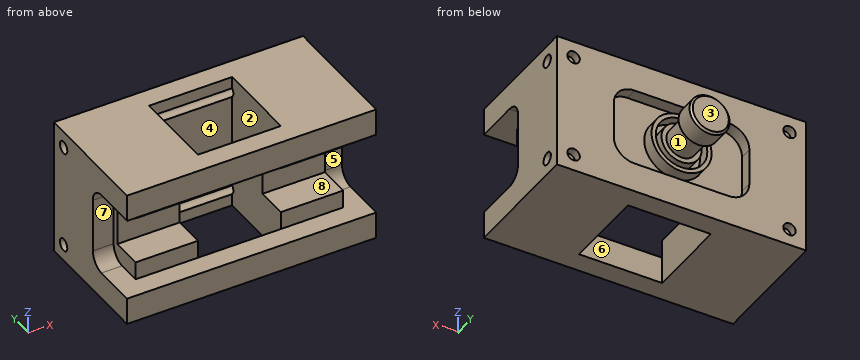
```python
from build123d import *

# Parameters (mm, degrees)
SKETCH1_W           = 120
SKETCH1_H           = 66
BOSS_EXTRUDE1_DEPTH = 60
SKETCH3_W           = 40
SKETCH3_H           = 20
CUT_EXTRUDE1_DEPTH  = 120
SKETCH4_W           = 40
SKETCH4_H           = 40
CUT_EXTRUDE2_DEPTH  = 120
SKETCH5_W           = 22.599154532
SKETCH5_H           = 30
CUT_EXTRUDE3_DEPTH  = 120
SKETCH6_R           = 3
CUT_EXTRUDE4_DEPTH  = 120
SKETCH7_W           = 40
SKETCH7_H           = 18
CUT_EXTRUDE5_DEPTH  = 10
SKETCH8_W           = 40
SKETCH8_H           = 18
CUT_EXTRUDE6_DEPTH  = 10
SKETCH9_W           = 65.307661508
SKETCH9_H           = 37.522692198
CUT_EXTRUDE7_DEPTH  = 6
FILLET1_R           = 10
SKETCH10_R          = 3
CUT_EXTRUDE8_DEPTH  = 4
FILLET2_R           = 7
SKETCH11_R          = 14.45708456
SKETCH11_R_2        = 12.407691548
BOSS_EXTRUDE2_DEPTH = 6
SKETCH12_R          = 9.667792976
BOSS_EXTRUDE3_DEPTH = 6
SKETCH13_R          = 7.310717913
BOSS_EXTRUDE4_DEPTH = 12
SKETCH14_R          = 9.667792976
BOSS_EXTRUDE5_DEPTH = 12
CHAMFER1_SIZE       = 2
CHAMFER2_SIZE       = 1


with BuildPart() as part:
    # Sketch1 → Boss-Extrude1 (new body)
    with BuildSketch(Plane(origin=(0, 0, 0), x_dir=(1, 0, 0), z_dir=(0, 1, 0))):
        Rectangle(SKETCH1_W, SKETCH1_H)
    extrude(amount=BOSS_EXTRUDE1_DEPTH)

    # Sketch3 → Cut-Extrude1 (cut)
    with BuildSketch(Plane(origin=(60, 0, 0), x_dir=(0, 0, -1), z_dir=(1, 0, 0))):
        Rectangle(SKETCH3_W, SKETCH3_H)
    extrude(amount=-CUT_EXTRUDE1_DEPTH, mode=Mode.SUBTRACT)

    # Sketch4 → Cut-Extrude2 (cut)
    with BuildSketch(Plane.XY.offset(33)):
        with Locations((0, 30)):
            Rectangle(SKETCH4_W, SKETCH4_H)
    extrude(amount=-CUT_EXTRUDE2_DEPTH, mode=Mode.SUBTRACT)

    # Sketch5 → Cut-Extrude3 (cut)
    with BuildSketch(Plane(origin=(60, 0, 0), x_dir=(0, 0, -1), z_dir=(1, 0, 0))):
        with Locations((0, 10)):
            Rectangle(SKETCH5_W, SKETCH5_H)
    extrude(amount=-CUT_EXTRUDE3_DEPTH, mode=Mode.SUBTRACT)

    # Sketch6 → Cut-Extrude4 (cut)
    with BuildSketch(Plane(origin=(60, 0, 0), x_dir=(0, 0, -1), z_dir=(1, 0, 0))):
        with Locations((-25, 52)):
            Circle(SKETCH6_R)
        with Locations((25, 52)):
            Circle(SKETCH6_R)
    extrude(amount=-CUT_EXTRUDE4_DEPTH, mode=Mode.SUBTRACT)

    # Sketch7 → Cut-Extrude5 (cut)
    with BuildSketch(Plane(origin=(60, 0, 0), x_dir=(0, 0, -1), z_dir=(1, 0, 0))):
        with Locations((0, 19)):
            Rectangle(SKETCH7_W, SKETCH7_H)
    extrude(amount=-CUT_EXTRUDE5_DEPTH, mode=Mode.SUBTRACT)

    # Sketch8 → Cut-Extrude6 (cut)
    with BuildSketch(Plane.ZY.offset(60)):
        with Locations((0, 19)):
            Rectangle(SKETCH8_W, SKETCH8_H)
    extrude(amount=-CUT_EXTRUDE6_DEPTH, mode=Mode.SUBTRACT)

    # Sketch9 → Cut-Extrude7 (cut)
    with BuildSketch(Plane(origin=(0, 60, 0), x_dir=(1, 0, 0), z_dir=(0, 1, 0))):
        Rectangle(SKETCH9_W, SKETCH9_H)
    extrude(amount=-CUT_EXTRUDE7_DEPTH, mode=Mode.SUBTRACT)

    # Fillet1
    fillet1_edges = [part.edges().sort_by_distance(p)[0] for p in [
        (32.653830754, 57, -18.761346099),
        (32.653830754, 57, 18.761346099),
        (-32.653830754, 57, 18.761346099),
        (-32.653830754, 57, -18.761346099),
    ]]
    fillet(fillet1_edges, radius=FILLET1_R)

    # Sketch10 → Cut-Extrude8 (cut)
    with BuildSketch(Plane(origin=(0, 60, 0), x_dir=(1, 0, 0), z_dir=(0, 1, 0))):
        with Locations(Location((-52, 25, 0), (0, 0, 270))):
            Circle(SKETCH10_R)
        with Locations(Location((52, 25, 0), (0, 0, 270))):
            Circle(SKETCH10_R)
        with Locations(Location((-52, -25, 0), (0, 0, 270))):
            Circle(SKETCH10_R)
        with Locations(Location((52, -25, 0), (0, 0, 270))):
            Circle(SKETCH10_R)
    extrude(amount=-CUT_EXTRUDE8_DEPTH, mode=Mode.SUBTRACT)

    # Fillet2
    fillet2_edges = [part.edges().sort_by_distance(p)[0] for p in [
        (55, 28, 20),
        (55, 28, -20),
        (-55, 28, -20),
        (-55, 28, 20),
    ]]
    fillet(fillet2_edges, radius=FILLET2_R)

    # Sketch11 → Boss-Extrude2 (add)
    with BuildSketch(Plane(origin=(0, 54, 0), x_dir=(1, 0, 0), z_dir=(0, 1, 0))):
        with Locations(Location((0, 0, 0), (0, 0, 270))):
            Circle(SKETCH11_R)
        with Locations(Location((0, 0, 0), (0, 0, 270))):
            Circle(SKETCH11_R_2, mode=Mode.SUBTRACT)
    extrude(amount=BOSS_EXTRUDE2_DEPTH)

    # Sketch12 → Boss-Extrude3 (add)
    with BuildSketch(Plane(origin=(0, 54, 0), x_dir=(1, 0, 0), z_dir=(0, 1, 0))):
        with Locations(Location((0, 0, 0), (0, 0, 270))):
            Circle(SKETCH12_R)
    extrude(amount=BOSS_EXTRUDE3_DEPTH)

    # Sketch13 → Boss-Extrude4 (add)
    with BuildSketch(Plane(origin=(0, 60, 0), x_dir=(1, 0, 0), z_dir=(0, 1, 0))):
        with Locations(Location((0, 0, 0), (0, 0, 270))):
            Circle(SKETCH13_R)
    extrude(amount=BOSS_EXTRUDE4_DEPTH)

    # Sketch14 → Boss-Extrude5 (add)
    with BuildSketch(Plane(origin=(0, 72, 0), x_dir=(1, 0, 0), z_dir=(0, 1, 0))):
        with Locations(Location((0, 0, 0), (0, 0, 270))):
            Circle(SKETCH14_R)
    extrude(amount=BOSS_EXTRUDE5_DEPTH)

    # Chamfer1
    chamfer1_edges = [part.edges().sort_by_distance(p)[0] for p in [
        (0, 72, -9.667792976),
    ]]
    chamfer(chamfer1_edges, length=CHAMFER1_SIZE)

    # Chamfer2
    chamfer2_edges = [part.edges().sort_by_distance(p)[0] for p in [
        (0, 84, -9.667792976),
    ]]
    chamfer(chamfer2_edges, length=CHAMFER2_SIZE)


solid = part.part
```
The listing builds one solid part. Answer for the finished solid, in the listing's coordinates (mm). Face numbers are marked on the shaded views. A direction names the side the tool comes from. Round coordinates to 2 decimals unless told otherwise and drop trailing zeros. Loops run counter-clockwise (first coordinate to the right, second up) from the corner with the lowest first, then second, coordinate; pieces in that order, holes last.
1) For the marked faces 5, 6, 7 and 8, determine the directions among +Z, -Z, +X, -X, +Y, -Y from which every point of the face is accessible in a straight line to the end or side of a thin tool.
Outcome:
face 5: +X, -Y
face 6: +Z, -Z
face 7: -X, -Y
face 8: +X, -X, -Y
2) Consider line 1 (X direction, y = 58, z = 25); line 2 (Z direction, x = -48, y = 21); line 3 (Y direction, x = 4, z = 25). Determine where each line is inside the solid, lowest interval first.
Outcome:
line 1: x = -60 to -55, -49 to 49, 55 to 60
line 2: z = -33 to -11.3, 11.3 to 33
line 3: y = 0 to 10, 55 to 60
3) Given P1, Ø3, axis at x = -37.5, z = 2.5, coming from the -Y side; P2, Ø3, axis at x = 51, z = -26.5, coming from the +Y side; P3, Ø12, axis at y = 68, z = 10.5, coming from the -X side, each flat-ended and moving along its own axis, determine where each tip first touches the part or whether it passes through.
Outcome:
P1: stops at y = 25
P2: stops at y = 60
P3: stops at x = -5.76
4) A cutting plane is placed at D-D on x = -37.5. Determine the outline of the cut face in (y, z), plus the area to 3 significant figures.
Outcome:
outline: (0, -33) - (60, -33) - (60, 33) - (0, 33) - (0, 20) - (10, 20) - (10, 11.3) - (25, 11.3) - (25, -11.3) - (10, -11.3) - (10, -20) - (0, -20) - close; hole circle Ø6 at (52, -25); hole circle Ø6 at (52, 25)
area: 3,160 mm2
5) For a pull along X with two mould halves and no side action, classify the marked faces 1, 2, 3 and 4 as released by +X, released by -X, zero draft, split by the parting line, or undercut.
Outcome:
face 1: split by the parting line
face 2: undercut
face 3: zero draft
face 4: undercut
6) A cutting plane is placed at A-A on y = 42. Determine the outline of the cut face in (x, z), plus the area to 3 significant figures.
Outcome:
outline: (-60, -33) - (-20, -33) - (-20, 33) - (-60, 33) - close; (20, -33) - (60, -33) - (60, 33) - (20, 33) - close
area: 5,280 mm2
7) A cutting plane is placed at C-C on y = 17. Determine the outline of the cut face in (x, z), plus the area to 3 significant figures.
Outcome:
outline: (-60, -33) - (-20, -33) - (-20, -11.3) - (-50, -11.3) - (-50, -20) - (-60, -20) - close; (-60, 20) - (-50, 20) - (-50, 11.3) - (-20, 11.3) - (-20, 33) - (-60, 33) - close; (20, -33) - (60, -33) - (60, -20) - (50, -20) - (50, -11.3) - (20, -11.3) - close; (20, 11.3) - (50, 11.3) - (50, 20) - (60, 20) - (60, 33) - (20, 33) - close
area: 3,120 mm2
8) A cutting plane is placed at B-B on z = -25. Determine the outline of the cut face in (x, y).
Outcome:
outline: (-60, 0) - (60, 0) - (60, 49) - (20, 49) - (20, 10) - (-20, 10) - (-20, 49) - (-60, 49) - close; (-60, 55) - (60, 55) - (60, 60) - (55, 60) - (55, 56) - (49, 56) - (49, 60) - (-49, 60) - (-49, 56) - (-55, 56) - (-55, 60) - (-60, 60) - close
